For this review, use the dimensioned drawing (mm, ordinates from the lowest corner) and the shaded views. Give positions to 0.01 mm unless a question says otherwise; leave off trailing zeros. Loops run counter-clockwise (first coordinate to the right, second up) from the corner with the lowest first, then second, coordinate; pieces in that order, holes last. Notation, with made-up numbers: (12, -40) - (25, -40) arc R13 ccw to (25, -24) - close; hole circle Ø6 at (-37, 87.25). An arc over 180 degrees is marked (long way). Write each question's results on one line, items separated by ' | '.
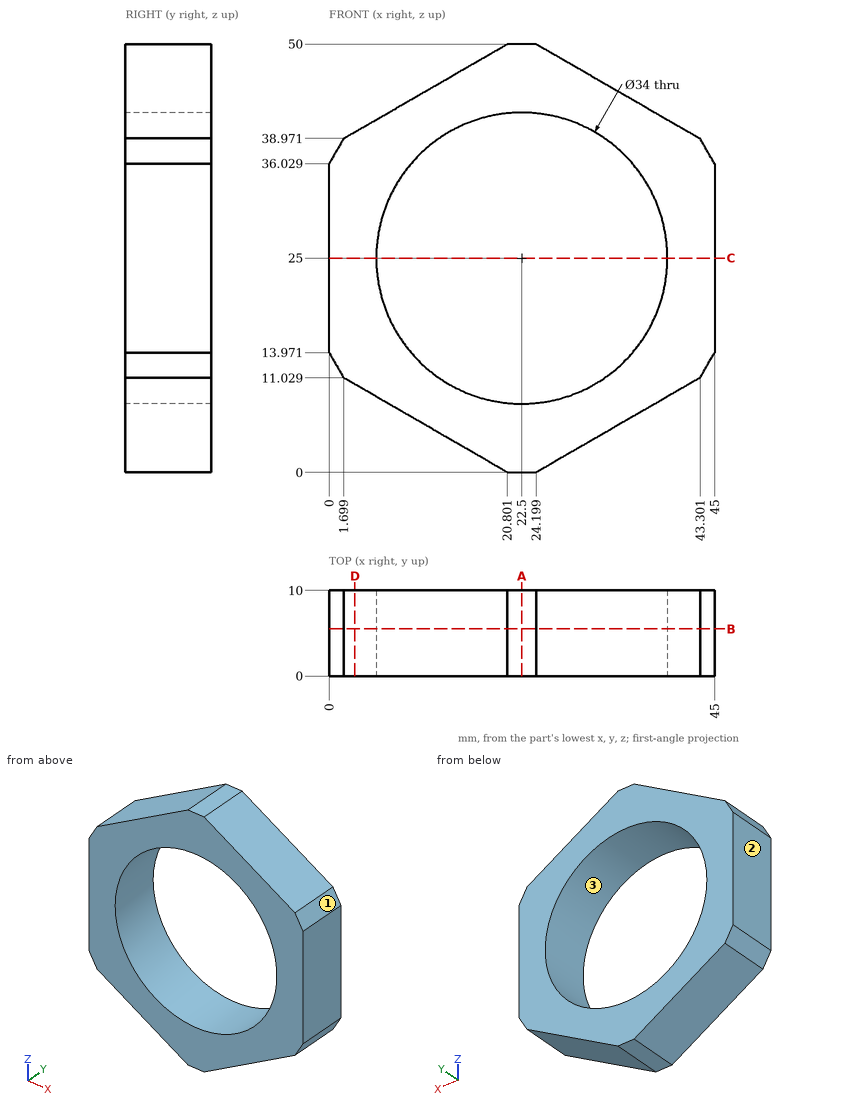
Item 1: We need section C-C on z = 25. Give the boundary of the cut face in (x, y).
Output values:
outline: (0, 0) - (5.5, 0) - (5.5, 10) - (0, 10) - close; (39.5, 0) - (45, 0) - (45, 10) - (39.5, 10) - close
Item 2: Wall thickness on probe 1 along Z at (x, y) = (22.5, 3.75); probe 2 along X at (y, z) = (5, 19) (1 decimal); probe 3 along X at (y, z) = (3, 24): over which ranges is each line inside the solid? List them lowest first.
Output values:
probe 1: z = 0 to 8, 42 to 50 | probe 2: x = 0 to 6.6, 38.4 to 45 | probe 3: x = 0 to 5.53, 39.47 to 45
Item 3: Draft analysis for pull direction X (two halves, no side actions). For the marked faces 1, 2 and 3, state which applies: +X half, -X half, draft (parallel to the pull), parting line (faces both ways), or undercut.
Output values:
face 1: +X half | face 2: -X half | face 3: undercut
Item 4: We need section B-B on y = 5.5. Give the boundary of the cut face in (x, z).
Output values:
outline: (0, 13.97) - (1.7, 11.03) - (20.8, 0) - (24.2, 0) - (43.3, 11.03) - (45, 13.97) - (45, 36.03) - (43.3, 38.97) - (24.2, 50) - (20.8, 50) - (1.7, 38.97) - (0, 36.03) - close; hole circle Ø34 at (22.5, 25)
Item 5: Clearance check with flat-ended pins moving along their axes: P1, Ø4, axis at x = 10, y = 2, coming from the -Z side; P2, Ø5, axis at y = 2.5, z = 11, coming from the -X side; P3, Ø3, axis at x = 31.5, y = 5, coming from the -Z side; P4, Ø1, axis at x = 37, z = 44.5, coming from the -Y side. State where each tip first meets the part, or that it passes through.
Output values:
P1: stops at z = 5.08 | P2: stops at x = 0.27 | P3: stops at z = 3.35 | P4: passes through
Item 6: We need section D-D on x = 3. Give the boundary of the cut face in (y, z), then the cut area to 3 significant figures.
Output values:
outline: (0, 10.28) - (10, 10.28) - (10, 39.72) - (0, 39.72) - close | area: 294 mm²
Item 7: We need section A-A on x = 22.5. Give the boundary of the cut face in (y, z), then the cut area to 3 significant figures.
Output values:
outline: (0, 0) - (10, 0) - (10, 8) - (0, 8) - close; (0, 42) - (10, 42) - (10, 50) - (0, 50) - close | area: 160 mm²
